from build123d import *

# Parameters (mm, degrees)
CUT_EXTRUDE1_REACH     = 42.398
SKETCH2_W              = 4
SKETCH2_H              = 9.816803941
M4_TAPPED_HOLE1_REACH  = 53.556
M4_TAPPED_HOLE1_BORE_R = 1.65


with BuildPart() as part:
    # Sketch1 → Revolve1 (revolve)
    with BuildSketch(Plane.XY, mode=Mode.PRIVATE) as revolve1_sk:
        Polygon((0, 10), (8, 10), (8, 15), (1.5, 15), (1.5, 28), (0, 28), align=None)
    revolve(revolve1_sk.sketch.rotate(Axis((0, 0, 0), (1, 0, 0)), 90), axis=Axis((0, 0, 0), (1, 0, 0)))

    # Sketch2 → Cut-Extrude1 (cut, up to next)
    with BuildSketch(Plane.ZY, mode=Mode.PRIVATE) as cut_extrude1_sk1:
        with Locations((0, 24.908401971)):
            Rectangle(SKETCH2_W, SKETCH2_H)
    cut_extrude1_tool1 = extrude(cut_extrude1_sk1.sketch, amount=-CUT_EXTRUDE1_REACH, mode=Mode.PRIVATE) & part.part
    add(cut_extrude1_tool1.solids().sort_by_distance((0, 24.908402, 0))[0], mode=Mode.SUBTRACT)

    # M4 Tapped Hole1 bore (on position points) → M4 Tapped Hole1 (cut, up to next)
    with BuildSketch(Plane(origin=(5, 0, -15), x_dir=(0, -1, 0), z_dir=(0, 0, -1)), mode=Mode.PRIVATE) as m4_tapped_hole1_sk1:
        Circle(M4_TAPPED_HOLE1_BORE_R)
    m4_tapped_hole1_tool1 = extrude(m4_tapped_hole1_sk1.sketch, amount=-M4_TAPPED_HOLE1_REACH, mode=Mode.PRIVATE) & part.part
    add(m4_tapped_hole1_tool1.solids().sort_by_distance((5, 0, -15))[0], mode=Mode.SUBTRACT)


solid = part.part
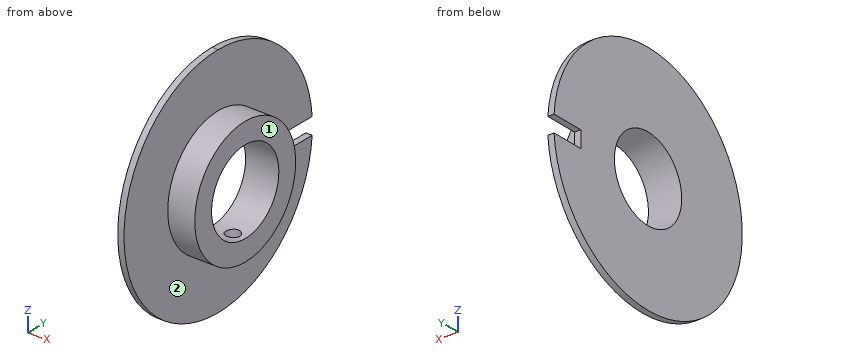
Could you check a few things on this model? Use its own coordinates, in mm. Face numbers are marked on the shaded views. A direction names the side the tool comes from. Coordinates: 2 decimals unless noted, no trailing zeros. Loops run counter-clockwise (first coordinate to the right, second up) from the corner with the lowest first, then second, coordinate; pieces in that order, holes last.
1. Imagine slicing it at A-A (z = 0). Please give me the cut outline in (x, y), and give its area (3 significant figures).
2. Imagine slicing it at C-C (x = 2.5). Please give me the cut outline in (y, z), and give its area (3 significant figures).
3. Imagine slicing it at D-D (y = 14). Please give me the cut outline in (x, z).
4. For the marked faces 1 and 2, which set-ups out of +Z, -Z, +X, -X, +Y, -Y let a thin tool reach every point of the face, with its end or its side?
5. I need wall thicknesses on L1, parallel to Y at x = 6.25, z = 0; L2, parallel to X at y = 0, z = -12.75; L3, parallel to X at y = -16.5, z = 21. Which ranges of each line are inside material? Lowest first, please.
6. For P1, Ø12, axis at y = -12, z = 15, coming from the -X side; P2, Ø1.5, axis at x = 1, z = 21.5, coming from the +Y side; P3, Ø1.2, axis at x = 0.5, y = 22.5, coming from the +Z side, each with a flat end and sliding along its axis, tell me the tip position at first contact or that it passes through.
7. Imagine slicing it at B-B (y = -8). Please give me the cut outline in (x, z).
Computed values:
1. outline: (0, -28) - (1.5, -28) - (1.5, -15) - (8, -15) - (8, -10) - (0, -10) - close; (0, 10) - (8, 10) - (8, 15) - (1.5, 15) - (1.5, 20) - (0, 20) - close
1. area: 107 mm2
2. outline: circle Ø30 at (0, 0); hole circle Ø20 at (0, 0)
2. area: 393 mm2
3. outline: (0, -24.25) - (1.5, -24.25) - (1.5, -5.39) - (8, -5.39) - (8, 5.39) - (1.5, 5.39) - (1.5, 24.25) - (0, 24.25) - close
4. face 1: +Z, -Z, +X, +Y, -Y
4. face 2: +X
5. L1: y = -15 to -10, 10 to 15
5. L2: x = 0 to 3.35, 6.65 to 8
5. L3: x = 0 to 1.5
6. P1: stops at x = 0
6. P2: stops at y = 18.8
6. P3: stops at z = 17.45
7. outline: (0, -26.83) - (1.5, -26.83) - (1.5, -12.69) - (8, -12.69) - (8, -6) - (0, -6) - close; (0, 6) - (8, 6) - (8, 12.69) - (1.5, 12.69) - (1.5, 26.83) - (0, 26.83) - close
